Geometry: final body of the model. Coordinates: model frame, mm. Face numbers are marked on the shaded views. A direction names the side the tool comes from. Give positions to 0.01 mm unless a question says otherwise; leave off trailing zeros. Loops run counter-clockwise (first coordinate to the right, second up) from the corner with the lowest first, then second, coordinate; pieces in that order, holes last. Notation, with made-up numbers: M -28,-34.75 L 7,-34.75 A7 ccw 7,-30.75 Z; hole C -34,73.25 d6. An arc over 180 degrees is marked long. Put each result on its own line as item: value.
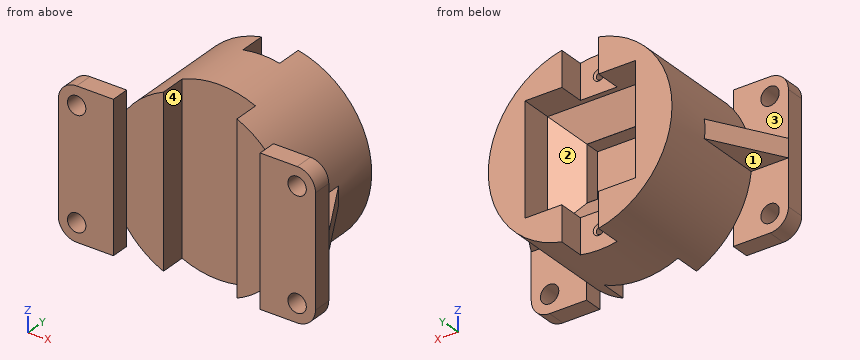
```python
from build123d import *

# Parameters (mm, degrees)
BASE_PLATE_SKETCH_R              = 5
BASE_PLATE_DEPTH                 = 10
BODY_CYLINDER_SKETCH_R           = 50
CYLINDRICAL_BODY_100_DEPTH       = 60
SQUARE_POCKET_60X60_DEPTH        = 17
LOWER_POCKET_DEPTH               = 17
DRAFTED_BOSS_SKETCH_W            = 30
DRAFTED_BOSS_SKETCH_H            = 30
DRAFTED_BOSS_DEPTH               = 9
DRAFTED_BOSS_DRAFT               = -58.93
SLOT_A_DEPTH                     = 34
INNER_BOSS_SKETCH_W              = 60
INNER_BOSS_SKETCH_H              = 60
INNER_BOSS_DEPTH                 = 44
SLOT_B_DEPTH                     = 34
CHANNEL_CUT_DEPTH                = 17
DRAFTED_CHANNEL_SKETCH_W         = 60
DRAFTED_CHANNEL_SKETCH_H         = 60
DRAFTED_CHANNEL_CUT_DEPTH        = 9
DRAFTED_CHANNEL_CUT_DRAFT        = -58.93
STEP_POCKET_SKETCH_W             = 20
STEP_POCKET_SKETCH_H             = 20
STEP_POCKET_DEPTH                = 14
PAD_HOLE_CHAMFER_SKETCH_R        = 3
PAD_HOLE_CHAMFER_DEPTH           = 1
PAD_HOLE_CHAMFER_DRAFT           = -45
PAD_HOLE_CHAMFER_PROFILE_2_DEPTH = 1
PAD_HOLE_CHAMFER_PROFILE_2_DRAFT = -45
PAD_HOLE_SKETCH_R                = 2
PAD_HOLE_DEPTH                   = 10
LEFT_SUPPORT_RIB_REACH           = 112.905
LEFT_RIB_SKETCH_WALL_W           = 264.12201887
LEFT_RIB_SKETCH_WALL_H           = 10
RIGHT_SUPPORT_RIB_REACH          = 112.905
RIGHT_RIB_SKETCH_WALL_W          = 264.12201887
RIGHT_RIB_SKETCH_WALL_H          = 10
SIDE_CUT_A_DEPTH                 = 126
SIDE_CUT_B_DEPTH                 = 202


with BuildPart() as part:
    # Base Plate Sketch → Base Plate (new body)
    with BuildSketch(Plane(origin=(0, 0, 0), x_dir=(1, 0, 0), z_dir=(0, 1, 0))):
        with BuildLine():
            Line((-60, -40), (0, -40))
            Line((0, -40), (60, -40))
            ThreePointArc((60, -40), (67.071067812, -37.071067812), (70, -30))
            Line((70, -30), (70, 0))
            Line((70, 0), (70, 30))
            ThreePointArc((70, 30), (67.071067812, 37.071067812), (60, 40))
            Line((60, 40), (-60, 40))
            ThreePointArc((-60, 40), (-67.071067812, 37.071067812), (-70, 30))
            Line((-70, 30), (-70, -30))
            ThreePointArc((-70, -30), (-67.071067812, -37.071067812), (-60, -40))
        make_face()
        with Locations(Location((-60, -30, 0), (0, 0, 270))):
            Circle(BASE_PLATE_SKETCH_R, mode=Mode.SUBTRACT)
        with Locations(Location((60, -30, 0), (0, 0, 270))):
            Circle(BASE_PLATE_SKETCH_R, mode=Mode.SUBTRACT)
        with Locations(Location((-60, 30, 0), (0, 0, 270))):
            Circle(BASE_PLATE_SKETCH_R, mode=Mode.SUBTRACT)
        with Locations(Location((60, 30, 0), (0, 0, 270))):
            Circle(BASE_PLATE_SKETCH_R, mode=Mode.SUBTRACT)
    extrude(amount=BASE_PLATE_DEPTH)

    # Body Cylinder Sketch → Cylindrical Body Ø100 (add)
    with BuildSketch(Plane(origin=(0, 10, 0), x_dir=(1, 0, 0), z_dir=(0, 1, 0))):
        with Locations(Location((0, 0, 0), (0, 0, 53.130102354))):
            Circle(BODY_CYLINDER_SKETCH_R)
    extrude(amount=CYLINDRICAL_BODY_100_DEPTH)

    # Square Pocket Sketch → Square Pocket 60x60 (cut)
    with BuildSketch(Plane(origin=(0, 70, 0), x_dir=(1, 0, 0), z_dir=(0, 1, 0))):
        Polygon((30, 0), (30, 30), (-30, 30), (-30, -30), (30, -30), align=None)
    extrude(amount=-SQUARE_POCKET_60X60_DEPTH, mode=Mode.SUBTRACT)

    # Lower Pocket Sketch → Lower Pocket (cut)
    with BuildSketch(Plane(origin=(0, 53, 0), x_dir=(1, 0, 0), z_dir=(0, 1, 0))):
        Polygon((15, 0), (15, 15), (-15, 15), (-15, -15), (15, -15), align=None)
    extrude(amount=-LOWER_POCKET_DEPTH, mode=Mode.SUBTRACT)


with BuildPart() as body_2:
    # Drafted Boss Sketch → Drafted Boss (with draft: the straight prism first)
    with BuildSketch(Plane(origin=(0, 53, 0), x_dir=(1, 0, 0), z_dir=(0, 1, 0))):
        Rectangle(DRAFTED_BOSS_SKETCH_W, DRAFTED_BOSS_SKETCH_H)
    extrude(amount=DRAFTED_BOSS_DEPTH)
    # Drafted Boss: the draft: its side faces are tilted about the plane it starts from
    drafted_boss_sides = [body_2.faces().sort_by_distance(p)[0] for p in [
        (-15, 57.5, 0),
        (0, 57.5, 15),
        (15, 57.5, 0),
        (0, 57.5, -15),
    ]]
    draft(drafted_boss_sides, Plane(origin=(0, 53, 0), x_dir=(1, 0, 0), z_dir=(0, 1, 0)), DRAFTED_BOSS_DRAFT)


with BuildPart() as slot_a_tool:
    # Slot A Sketch → Slot A (new body)
    with BuildSketch(Plane(origin=(0, 62, 0), x_dir=(1, 0, 0), z_dir=(0, 1, 0))):
        Polygon((15, 0), (15, 15), (-15, 15), (-15, -15), (15, -15), align=None)
    extrude(amount=-SLOT_A_DEPTH)


with BuildPart() as part_1:
    add(part.part)

    # Slot A: cut by slot_a_tool
    add(slot_a_tool.part, mode=Mode.SUBTRACT)



with BuildPart() as body_2_1:
    add(body_2.part)

    # Slot A: cut by slot_a_tool
    add(slot_a_tool.part, mode=Mode.SUBTRACT)


with BuildPart() as part_2:
    add(part_1.part)

    add(body_2_1.part)  # Inner Boss merges body 2
    # Inner Boss Sketch → Inner Boss (add)
    with BuildSketch(Plane(origin=(0, 70, 0), x_dir=(1, 0, 0), z_dir=(0, 1, 0))):
        Rectangle(INNER_BOSS_SKETCH_W, INNER_BOSS_SKETCH_H)
    extrude(amount=-INNER_BOSS_DEPTH)

    # Slot B Sketch → Slot B (cut)
    with BuildSketch(Plane(origin=(0, 70, 0), x_dir=(1, 0, 0), z_dir=(0, 1, 0))):
        Polygon((15, 0), (15, 15), (-15, 15), (-15, -15), (15, -15), align=None)
    extrude(amount=-SLOT_B_DEPTH, mode=Mode.SUBTRACT)

    # Channel Sketch → Channel Cut (cut)
    with BuildSketch(Plane(origin=(0, 70, 0), x_dir=(1, 0, 0), z_dir=(0, 1, 0))):
        Polygon((30, 0), (30, 30), (-30, 30), (-30, -30), (30, -30), align=None)
    extrude(amount=-CHANNEL_CUT_DEPTH, mode=Mode.SUBTRACT)


with BuildPart() as drafted_channel_cut_tool:
    # Drafted Channel Sketch → Drafted Channel Cut (with draft: the straight prism first)
    with BuildSketch(Plane(origin=(0, 53, 0), x_dir=(1, 0, 0), z_dir=(0, 1, 0))):
        Rectangle(DRAFTED_CHANNEL_SKETCH_W, DRAFTED_CHANNEL_SKETCH_H)
    extrude(amount=-DRAFTED_CHANNEL_CUT_DEPTH)
    # Drafted Channel Cut: the draft: its side faces are tilted about the plane it starts from
    drafted_channel_cut_sides = [drafted_channel_cut_tool.faces().sort_by_distance(p)[0] for p in [
        (-30, 48.5, 0),
        (0, 48.5, 30),
        (30, 48.5, 0),
        (0, 48.5, -30),
    ]]
    draft(drafted_channel_cut_sides, Plane(origin=(0, 53, 0), x_dir=(1, 0, 0), z_dir=(0, 1, 0)), DRAFTED_CHANNEL_CUT_DRAFT)


with BuildPart() as part_3:
    add(part_2.part)

    # Drafted Channel Cut: cut by drafted_channel_cut_tool
    add(drafted_channel_cut_tool.part, mode=Mode.SUBTRACT)

    # Step Pocket Sketch → Step Pocket (cut)
    with BuildSketch(Plane(origin=(0, 70, 0), x_dir=(1, 0, 0), z_dir=(0, 1, 0))):
        with Locations((0, -40)):
            Rectangle(STEP_POCKET_SKETCH_W, STEP_POCKET_SKETCH_H)
        Polygon((0, 30), (10, 30), (10, 50), (-10, 50), (-10, 30), align=None)
    extrude(amount=-STEP_POCKET_DEPTH, mode=Mode.SUBTRACT)


with BuildPart() as pad_hole_chamfer_tool:
    # Pad Hole Chamfer Sketch → Pad Hole Chamfer (with draft: the straight prism first)
    with BuildSketch(Plane(origin=(0, 56, 0), x_dir=(1, 0, 0), z_dir=(0, 1, 0))):
        with Locations((0, -39.494897428)):
            Circle(PAD_HOLE_CHAMFER_SKETCH_R)
    extrude(amount=-PAD_HOLE_CHAMFER_DEPTH)
    # Pad Hole Chamfer: the draft: its side faces are tilted about the plane it starts from
    pad_hole_chamfer_sides = [pad_hole_chamfer_tool.faces().sort_by_distance(p)[0] for p in [
        (-3, 55.5, 39.494897428),
    ]]
    draft(pad_hole_chamfer_sides, Plane(origin=(0, 56, 0), x_dir=(1, 0, 0), z_dir=(0, 1, 0)), PAD_HOLE_CHAMFER_DRAFT)


with BuildPart() as part_4:
    add(part_3.part)

    # Pad Hole Chamfer: cut by pad_hole_chamfer_tool
    add(pad_hole_chamfer_tool.part, mode=Mode.SUBTRACT)


with BuildPart() as pad_hole_chamfer_profile_2_tool:
    # Pad Hole Chamfer Sketch → Pad Hole Chamfer profile 2 (with draft: the straight prism first)
    with BuildSketch(Plane(origin=(0, 56, 0), x_dir=(1, 0, 0), z_dir=(0, 1, 0))):
        with Locations((0, 39.494897428)):
            Circle(PAD_HOLE_CHAMFER_SKETCH_R)
    extrude(amount=-PAD_HOLE_CHAMFER_PROFILE_2_DEPTH)
    # Pad Hole Chamfer profile 2: the draft: its side faces are tilted about the plane it starts from
    pad_hole_chamfer_profile_2_sides = [pad_hole_chamfer_profile_2_tool.faces().sort_by_distance(p)[0] for p in [
        (-3, 55.5, -39.494897428),
    ]]
    draft(pad_hole_chamfer_profile_2_sides, Plane(origin=(0, 56, 0), x_dir=(1, 0, 0), z_dir=(0, 1, 0)), PAD_HOLE_CHAMFER_PROFILE_2_DRAFT)


with BuildPart() as part_5:
    add(part_4.part)

    # Pad Hole Chamfer profile 2: cut by pad_hole_chamfer_profile_2_tool
    add(pad_hole_chamfer_profile_2_tool.part, mode=Mode.SUBTRACT)

    # Pad Hole Sketch → Pad Hole (cut)
    with BuildSketch(Plane(origin=(0, 55, 0), x_dir=(1, 0, 0), z_dir=(0, 1, 0))):
        with Locations(Location((0, 39.494897428, 0), (0, 0, 270))):
            Circle(PAD_HOLE_SKETCH_R)
        with Locations(Location((0, -39.494897428, 0), (0, 0, 270))):
            Circle(PAD_HOLE_SKETCH_R)
    extrude(amount=-PAD_HOLE_DEPTH, mode=Mode.SUBTRACT)

    # Left Rib Sketch wall → Left Support Rib (add, up to next)
    with BuildSketch(Plane(origin=(-60, 27.5, 0), x_dir=(-0.496138938357, -0.868243142124, 0), z_dir=(0.868243142124, -0.496138938357, 0)), mode=Mode.PRIVATE) as left_support_rib_sk1:
        Rectangle(LEFT_RIB_SKETCH_WALL_W, LEFT_RIB_SKETCH_WALL_H)
    left_support_rib_tool1 = extrude(left_support_rib_sk1.sketch, amount=LEFT_SUPPORT_RIB_REACH, mode=Mode.PRIVATE) - part_5.part
    add(left_support_rib_tool1.solids().sort_by_distance((-60, 27.5, 0))[0])

    # Right Rib Sketch wall → Right Support Rib (add, up to next)
    with BuildSketch(Plane(origin=(60, 27.5, 0), x_dir=(0.496138938357, -0.868243142124, 0), z_dir=(0.868243142124, 0.496138938357, 0)), mode=Mode.PRIVATE) as right_support_rib_sk1:
        Rectangle(RIGHT_RIB_SKETCH_WALL_W, RIGHT_RIB_SKETCH_WALL_H)
    right_support_rib_tool1 = extrude(right_support_rib_sk1.sketch, amount=-RIGHT_SUPPORT_RIB_REACH, mode=Mode.PRIVATE) - part_5.part
    add(right_support_rib_tool1.solids().sort_by_distance((60, 27.5, 0))[0])

    # Side Cut A Sketch → Side Cut A (cut)
    with BuildSketch(Plane.XY.offset(50)):
        Polygon((0, 10), (-40, 10), (-40, 0), (39.874685928, 0), (39.874685928, 10), align=None)
    extrude(amount=-SIDE_CUT_A_DEPTH, mode=Mode.SUBTRACT)

    # Side Cut B Sketch → Side Cut B (cut)
    with BuildSketch(Plane.XY.offset(50)):
        Polygon((0, 0), (20, 0), (20, 24), (-20, 24), (-20, 0), align=None)
    extrude(amount=-SIDE_CUT_B_DEPTH, mode=Mode.SUBTRACT)


solid = part_5.part
```
Item 1: Set-up query: the marked faces 1, 2, 3 and 4. Return all of +Z, -Z, +X, -X, +Y, -Y with unobstructed straight access to the full face (end or side cutting, diameter ignored); none if empty.
Output values:
face 1: -Z, -X, +Y
face 2: +Y
face 3: +Z, -X, +Y
face 4: +Z, -Z, -Y
Item 2: Section A-A on y = 64.5. Output: boundary loops of the cut face in (x, z).
Output values:
outline: M -30,-30 L -30,30 L -10,30 L -10,48.99 A50 ccw -10,-48.99 L -10,-30 Z; M 10,-48.99 A50 ccw 10,48.99 L 10,30 L 30,30 L 30,-30 L 10,-30 Z
Item 3: Section C-C on z = 0. Output: boundary loops of the cut face in (x, y), then the cut area to 3 significant figures.
Output values:
outline: M -70,0 L -40,0 L -40,10 L -20,10 L -20,24 L 20,24 L 20,10 L 39.87,10 L 39.87,0 L 70,0 L 70,10 L 50,45 L 50,70 L 30,70 L 30,53 L 15.06,44 L 15,44 L 15,36 L -15,36 L -15,44 L -15.06,44 L -30,53 L -30,70 L -50,70 L -50,45 L -70,10 Z
area: 5,080 mm²
Item 4: Section D-D on y = 50.5. Output: boundary loops of the cut face in (x, z), then the cut area to 3 significant figures.
Output values:
outline: C 0,0 d100; hole M -25.85,-25.85 L 25.85,-25.85 L 25.85,25.85 L -25.85,25.85 Z; hole C 0,-39.49 d4; hole C 0,39.49 d4
area: 5,160 mm²
Item 5: Line query: probe 1 along X at (y, z) = (5.25, 30); probe 2 along Z at (x, y) = (0, 48.5); probe 3 along X at (y, z) = (4, -8.5). Output: solid intervals per line, ascending. Write a range as [from, to].
Output values:
probe 1: [-70, -65], [-55, -40], [39.87, 55], [65, 70]
probe 2: [-50, -41.49], [-37.49, -22.53], [22.53, 37.49], [41.49, 50]
probe 3: [-70, -40], [39.87, 70]
Item 6: Pin query (flat end, axial travel): pin 1 Ø8 at (x, y) = (52, 4.5) entering from -Z; pin 2 Ø1 at (x, y) = (2, 40) entering from +Z; pin 3 Ø24 at (x, z) = (3.5, -0.5) entering from +Y. Return the tip coordinate at first contact, or that it passes through.
Output values:
pin 1: z = -40
pin 2: z = 49.98
pin 3: y = 44.26
Item 7: Section B-B on x = 0. Output: boundary loops of the cut face in (y, z).
Output values:
outline: M 24,-50 L 56,-50 L 56,-42.49 L 55,-41.49 L 45,-41.49 L 45,-37.49 L 55,-37.49 L 56,-36.49 L 56,-30 L 53,-30 L 44,-15.06 L 44,-15 L 36,-15 L 36,15 L 44,15 L 44,15.06 L 53,30 L 56,30 L 56,36.49 L 55,37.49 L 45,37.49 L 45,41.49 L 55,41.49 L 56,42.49 L 56,50 L 24,50 Z
